```python
from build123d import *

# Parameters (mm, degrees)
BOSS_EXTRUDE1_DEPTH = 6
CHAMFER1_SIZE       = 20


with BuildPart() as part:
    # Sketch1 → Boss-Extrude1 (new, symmetric)
    with BuildSketch(Plane(origin=(0, 0, 0), x_dir=(1, 0, 0), z_dir=(0, 1, 0))):
        Polygon((-20, 20), (-20, 350), (20, 350), (90, 60), (90, 0), (0, 0), (-20, 0), align=None)
    extrude(amount=BOSS_EXTRUDE1_DEPTH, both=True)

    # Chamfer1
    chamfer1_edges = [part.edges().sort_by_distance(p)[0] for p in [
        (-20, 0, 0),
    ]]
    chamfer(chamfer1_edges, length=CHAMFER1_SIZE)


solid = part.part
```
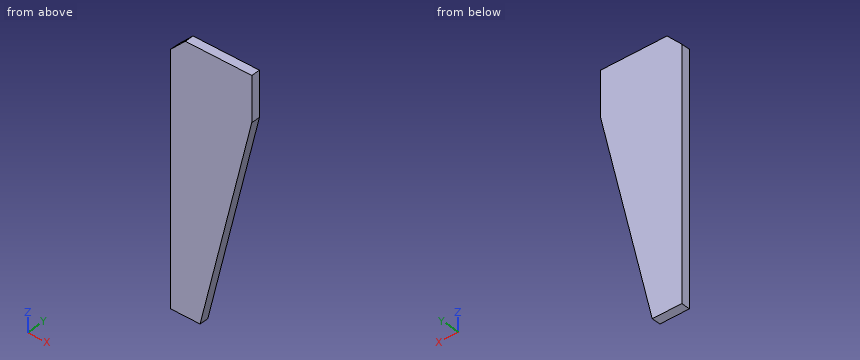
Could you check a few things on this model? Use its own coordinates, in mm. Round coordinates to 2 decimals unless told otherwise and drop trailing zeros. Loops run counter-clockwise (first coordinate to the right, second up) from the corner with the lowest first, then second, coordinate; pieces in that order, holes last.
Q1. I want a section at C-C (z = -191). Write out the boundary of the cut face in (x, y), and give its area (3 significant figures).
Q2. Please list where these lines run through material, in increasing order: L1, parallel to Z at x = -6, y = -3.75; L2, parallel to X at y = -3.5, z = -132.5; L3, parallel to X at y = 2, z = -126.5.
Q3. For P1, Ø5, axis at y = 4.5, z = -148, coming from the +X side, with a flat end and sliding along its axis, tell me the tip position at first contact or that it passes through.
Q4. I want a section at B-B (x = 72.5). Write out the boundary of the cut face in (y, z).
Q5. I want a section at A-A (y = 4). Write out the boundary of the cut face in (x, z), and give its area (4 significant figures).
Answer below:
1. outline: (-20, -6) - (58.38, -6) - (58.38, 6) - (-20, 6) - close
1. area: 941 mm2
2. L1: z = -350 to -6
2. L2: x = -20 to 72.5
2. L3: x = -20 to 73.95
3. P1: stops at x = 69.36
4. outline: (-6, -132.5) - (6, -132.5) - (6, 0) - (-6, 0) - close
5. outline: (-20, -350) - (20, -350) - (90, -60) - (90, 0) - (0, 0) - (-20, -20) - close
5. area: 28,150 mm2
